Input: part model. Units: mm. Frame: model coordinates. A direction names the side the tool comes from. Give positions to 0.01 mm unless a question says otherwise; leave off trailing zeros. Loops run counter-clockwise (first coordinate to the right, second up) from the corner with the lowest first, then second, coordinate; pieces in that order, holes last. Notation, with made-up numbers: (29, 59) - (73, 59) arc R18 ccw to (73, 76) - close; hole circle Ø4 at (-6.5, 57.5). An arc over 180 degrees is marked (long way). One line per item, written item: value.
from build123d import *

# Parameters (mm, degrees)
BOSS_EXTRUDE1_DEPTH = 8


with BuildPart() as part:
    # Sketch1 → Boss-Extrude1 (new body)
    with BuildSketch(Plane.XY):
        with BuildLine():
            Line((-194.542584235, 40.149199278), (-207.290309428, 40.149199278))
            ThreePointArc((-207.290309428, 40.149199278), (-218.290309428, 51.149199278), (-229.290309428, 40.149199278))
            Line((-229.290309428, 40.149199278), (-242.038034621, 40.149199278))
            Line((-242.038034621, 40.149199278), (-242.038034621, 99.149199278))
            Line((-242.038034621, 99.149199278), (-229.288034621, 99.149199278))
            Line((-229.288034621, 99.149199278), (-229.288034621, 91.149199278))
            Line((-229.288034621, 91.149199278), (-207.288034621, 91.149199278))
            Line((-207.288034621, 91.149199278), (-207.288034621, 99.149199278))
            Line((-207.288034621, 99.149199278), (-194.542584235, 99.149199278))
            Line((-194.542584235, 99.149199278), (-194.542584235, 40.149199278))
        make_face()
    extrude(amount=BOSS_EXTRUDE1_DEPTH)


solid = part.part
Item 1: Access query for faces 5 (the face through (-229.288, 95, 4)), 6 (the face through (-201, 40.149, 4)). Directions: +Z, -Z, +X, -X, +Y, -Y. A direction counts if a zero-diameter tool reaches every point of the face in a straight line with its end or side. Return the directions, or none.
Verdict:
face 5: +Z, -Z, +Y
face 6: +Z, -Z, +X, -X, -Y
Item 2: Material intervals for L1, parallel to X at y = 95, z = 7; L2, parallel to Y at x = -218, z = 6; L3, parallel to Y at x = -209, z = 6.5, sorted ascending.
Verdict:
L1: x = -242.04 to -229.29, -207.29 to -194.54
L2: y = 51.15 to 91.15
L3: y = 46.04 to 91.15
Item 3: Draft query along X for faces 1 (the face through (-218, 70, 8)), 2 (the face through (-194.543, 70, 4)), 3 (the face through (-218, 91.149, 4)), 4 (the face through (-242.038, 69, 4)). Return one class per face: pulls with the +X half, pulls with the -X half, needs draft (parallel to the pull), parting line crosses it, or undercut.
Verdict:
face 1: needs draft
face 2: pulls with the +X half
face 3: undercut
face 4: pulls with the -X half
Item 4: Pin query (flat end, axial travel): P1, Ø3, axis at x = -214.5, z = 6.5, coming from the +Y side. Return the tip coordinate at first contact, or that it passes through.
Verdict:
P1: stops at y = 91.15
Item 5: Section A-A, the plane y = 50.5. Output: boundary loops of the cut face in (x, z), and give its area (3 significant figures).
Verdict:
outline: (-242.04, 0) - (-222.01, 0) - (-222.01, 8) - (-242.04, 8) - close; (-214.57, 0) - (-194.54, 0) - (-194.54, 8) - (-214.57, 8) - close
area: 320 mm^2
Item 6: Section B-B, the plane z = 5.25. Output: boundary loops of the cut face in (x, y).
Verdict:
outline: (-242.04, 40.15) - (-229.29, 40.15) arc R11 cw to (-207.29, 40.15) - (-194.54, 40.15) - (-194.54, 99.15) - (-207.29, 99.15) - (-207.29, 91.15) - (-229.29, 91.15) - (-229.29, 99.15) - (-242.04, 99.15) - close
Item 7: Section D-D, the plane x = -224.5. Output: boundary loops of the cut face in (y, z).
Verdict:
outline: (49.23, 0) - (91.15, 0) - (91.15, 8) - (49.23, 8) - close
Item 8: Section C-C, the plane x = -213.5. Output: boundary loops of the cut face in (y, z).
Verdict:
outline: (50.05, 0) - (91.15, 0) - (91.15, 8) - (50.05, 8) - close
